```python
from build123d import *

# Parameters (mm, degrees)
HEX_PROFILE_20AF_R     = 5
HEX_NUT_BODY_6MM_DEPTH = 3


with BuildPart() as part:
    # Hex Profile 20AF → Hex Nut Body 6mm (new, symmetric)
    with BuildSketch(Plane.XY):
        Polygon((11.547005384, 0), (5.773502692, 10), (-5.773502692, 10), (-11.547005384, 0), (-5.773502692, -10), (5.773502692, -10), align=None)
        Circle(HEX_PROFILE_20AF_R, mode=Mode.SUBTRACT)
    extrude(amount=HEX_NUT_BODY_6MM_DEPTH, both=True)

    # Edge Chamfer Profile → Edge Chamfer Cut (revolve, cut)
    with BuildSketch(Plane(origin=(0, 0, 0), x_dir=(1, 0, 0), z_dir=(0, 1, 0))):
        with BuildLine():
            Line((10.547005384, 3), (11.547005384, 3))
            Line((11.547005384, 3), (11.547005384, 2))
            ThreePointArc((11.547005384, 2), (11.138343291, 2.591337907), (10.547005384, 3))
        make_face()
    edge_chamfer_cut = revolve(axis=Axis((0, 0, -5.076869621), (0, 0, 1)), mode=Mode.SUBTRACT)

    # Edge Chamfer Mirror: Edge Chamfer Cut across plane
    add(edge_chamfer_cut.mirror(Plane.XY), mode=Mode.SUBTRACT)


solid = part.part
```
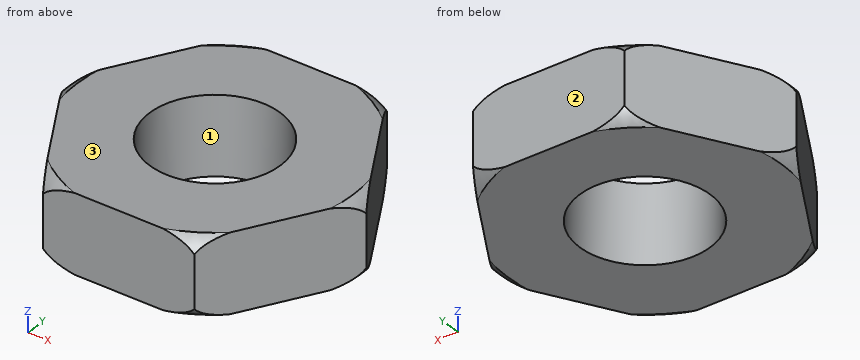
CAD build for the part. Positions are in the model's coordinates, mm. Face numbers are marked on the shaded views. Round coordinates to 2 decimals unless told otherwise and drop trailing zeros. Order: outer loops, then holes, each group sorted by start corner. A loop starts at its lowest first (then second) coordinate and runs counter-clockwise, first axis right, second up.
Q1. Slice it at C-C (z = -1.5). Write the cut outline in (x, y), and give its area (3 significant figures).
Q2. Slice it at B-B (y = -3.75). Write the cut outline in (x, z), and give its area (3 significant figures).
Q3. Two-plate mould, pull along Y, no slides. Class the marked faces 1, 2 and 3: pulls with the +Y half, pulls with the -Y half, needs draft (parallel to the pull), parting line crosses it, or undercut.
Q4. Slice it at D-D (x = 9.25). Write the cut outline in (y, z), and give its area (3 significant figures).
Q5. Wall check: L1, parallel to Y at x = 0, z = 1.65; L2, parallel to X at y = 3.5, z = 1; L3, parallel to Y at x = -1, z = 1.5. Give the ranges that are in metal, low to high.
Q6. Drop flat-ended pins along their axis: pin 1 (8 mm diameter, centred on x = 3, y = 2.5, fed in from +Z); pin 2 (1 mm diameter, centred on y = 2.5, z = 1, fed in from -X); pin 3 (2 mm diameter, centred on y = 3, z = -1, fed in from +X); pin 4 (2 mm diameter, centred on y = 4, z = 1, fed in from +X). Give the stop position or say it passes through.
Q7. Slice it at A-A (x = 0). Write the cut outline in (y, z).
Results below:
1. outline: (-11.55, 0) - (-5.77, -10) - (5.77, -10) - (11.55, 0) - (5.77, 10) - (-5.77, 10) - close; hole circle Ø10 at (0, 0)
1. area: 268 mm2
2. outline: (-9.38, -3) - (-3.31, -3) - (-3.31, 3) - (-9.38, 3) - close; (3.31, -3) - (9.38, -3) - (9.38, 3) - (3.31, 3) - close
2. area: 72.9 mm2
3. face 1: undercut
3. face 2: pulls with the +Y half
3. face 3: needs draft
4. outline: (-3.98, -3) - (3.98, -3) - (3.98, 3) - (-3.98, 3) - close
4. area: 47.7 mm2
5. L1: y = -10 to -5, 5 to 10
5. L2: x = -9.53 to -3.57, 3.57 to 9.53
5. L3: y = -10 to -4.9, 4.9 to 10
6. pin 1: stops at z = 3
6. pin 2: stops at x = -10.39
6. pin 3: stops at x = 10.39
6. pin 4: stops at x = 9.81
7. outline: (-10, -3) - (-5, -3) - (-5, 3) - (-10, 3) - close; (5, -3) - (10, -3) - (10, 3) - (5, 3) - close
